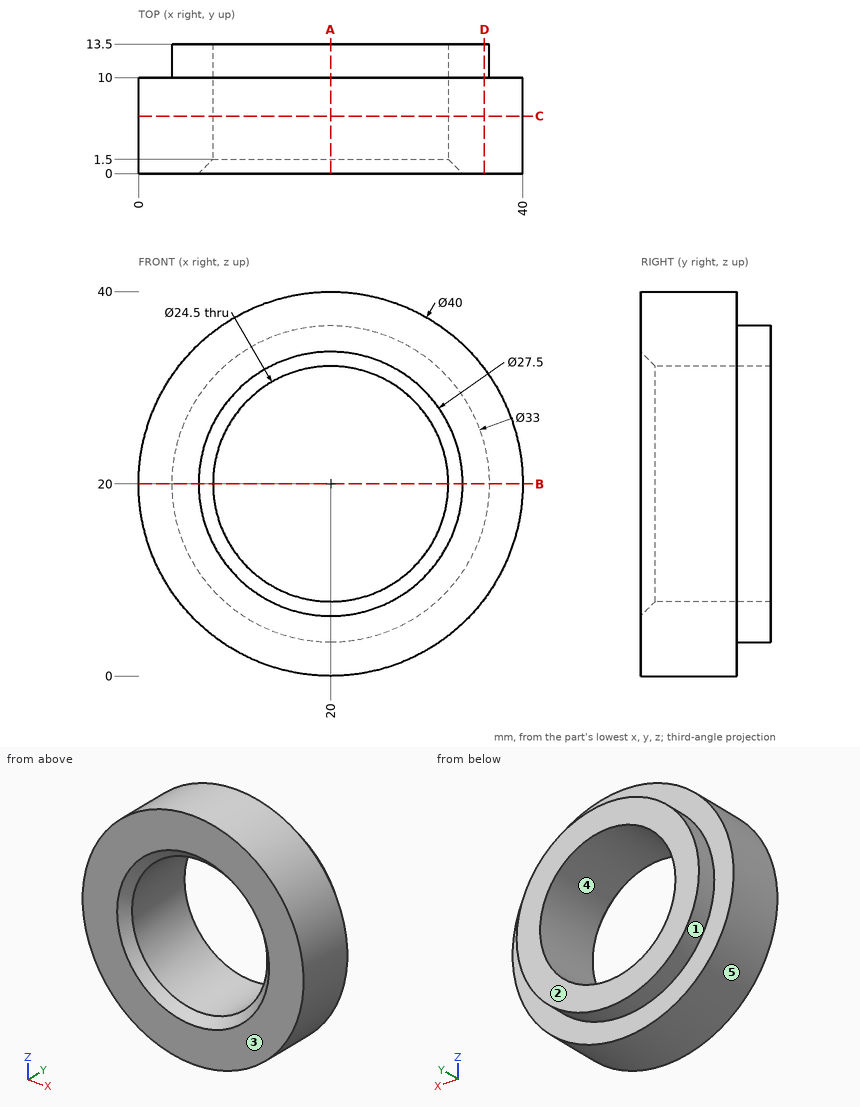
Answer from the drawing. Dimensions are ordinates in mm from the lowest x, y and z of the part. A direction names the side the tool comes from. Round coordinates to 2 decimals unless told otherwise and drop trailing zeros. Order: outer loops, then holes, each group sorted by start corner. A loop starts at its lowest first (then second) coordinate and runs counter-clockwise, first axis right, second up. Notation, with made-up numbers: (34.25, 31.25) - (47.25, 31.25) arc R30 ccw to (47.25, 57.25) - close; hole circle Ø1 at (4.25, -15.75). An arc over 180 degrees is marked (long way). Put each result on its own line as item: value. Start each with the question number.
(1) Find section A-A (x = 20). Give the vertices of the cut face in (y, z).
(2) For the marked faces 1 and 2, determine the directions among +Z, -Z, +X, -X, +Y, -Y from which every point of the face is accessible in a straight line to the end or side of a thin tool.
(3) Straight lines are drawn through the part: probe 1 along X at (y, z) = (4.5, 20); probe 2 along X at (y, z) = (11, 20); probe 3 along Y at (x, z) = (3, 11). For each, find the intervals that lie inside material, in ascending order. Write a range as from..to.
(4) Find section C-C (y = 6). Give the vertices of the cut face in (x, z).
(5) Find section D-D (x = 36). Give the vertices of the cut face in (y, z).
(6) Find section B-B (z = 20). Give the vertices of the cut face in (x, y).
(7) Determine the mould class of the marked faces 3, 4 and 5 for opening direction Z: released by +Z, released by -Z, zero draft, split by the parting line, or undercut.
(8) Given P1, Ø5, axis at y = 12, z = 23.5, coming from the -X side; P2, Ø8, axis at y = 4.5, z = 20.5, coming from the -X side; P3, Ø5, axis at x = 13.5, y = 5.5, coming from the +Z side, each flat-ended and moving along its own axis, determine where each tip first touches the part or whether it passes through.
Reply:
1. outline: (0, 0) - (10, 0) - (10, 3.5) - (13.5, 3.5) - (13.5, 7.75) - (1.5, 7.75) - (0, 6.25) - close; (0, 33.75) - (1.5, 32.25) - (13.5, 32.25) - (13.5, 36.5) - (10, 36.5) - (10, 40) - (0, 40) - close
2. face 1: +Y
2. face 2: +Z, -Z, +X, -X, +Y
3. probe 1: 0..7.75, 32.25..40
3. probe 2: 3.5..7.75, 32.25..36.5
3. probe 3: 0..10
4. outline: circle Ø40 at (20, 20); hole circle Ø24.5 at (20, 20)
5. outline: (0, 8) - (10, 8) - (10, 15.97) - (13.5, 15.97) - (13.5, 24.03) - (10, 24.03) - (10, 32) - (0, 32) - close
6. outline: (0, 0) - (6.25, 0) - (7.75, 1.5) - (7.75, 13.5) - (3.5, 13.5) - (3.5, 10) - (0, 10) - close; (32.25, 1.5) - (33.75, 0) - (40, 0) - (40, 10) - (36.5, 10) - (36.5, 13.5) - (32.25, 13.5) - close
7. face 3: zero draft
7. face 4: undercut
7. face 5: split by the parting line
8. P1: x = 0.1
8. P2: x = 0
8. P3: z = 39.6
